Verification items for the finished model (mm, model axes). Face numbers are marked on the shaded views. Coordinates: 2 decimals unless noted, no trailing zeros. Loops run counter-clockwise (first coordinate to the right, second up) from the corner with the lowest first, then second, coordinate; pieces in that order, holes last. Notation, with made-up numbers: (10.25, 48.25) - (51.25, 48.25) arc R32 cw to (51.25, 85.25) - close; hole circle Ø11 at (26, -15). An arc over 180 degrees is marked (long way). Answer as CSV lines item,"result". Start each with the question number.
1. Release check for a two-part mould opening along Z. For the marked faces 1 and 2 record: pulls with the +Z half, pulls with the -Z half, needs draft (parallel to the pull), parting line crosses it, or undercut.
2. Cross-section at B-B (z = 637). Enter the section's corners in (x, y).
3. Cross-section at A-A (y = 382). Enter the section's corners in (x, z).
4. Gauge pin test, flat ends, axial feed: P1, Ø4, axis at x = 76.5, z = 706, coming from the +Y side; P2, Ø11.5, axis at x = 16, z = 1563, coming from the -Y side; P3, Ø7, axis at y = 16, z = 1263, coming from the +X side; P4, Ø0.6, axis at x = 68.5, z = 1, coming from the +Y side. Record the tip position at first contact, or that the pin passes through.
5. Material ranges on line 1 (Z direction, x = 16, y = 479.25); line 2 (Y direction, x = 16, z = 0.55); line 3 (Y direction, x = 16, z = 2004), recorded low to high. Write a range as [from, to].
6. Cross-section at C-C (y = 87.5). Enter the section's corners in (x, z).
```python
from build123d import *

# Parameters (mm, degrees)
EXTRUDE_1_DEPTH     = 2005
EXTRUDE_1_2_DEPTH   = 28
EXTRUDE_2_DEPTH     = 28
SKETCH_5_W          = 120
SKETCH_5_H          = 2
EXTRUDE_3_DEPTH     = 165
SKETCH_7_R          = 4.5
CUT_EXTRUDE_2_DEPTH = 10
SKETCH_8_R          = 4.5
CUT_EXTRUDE_3_DEPTH = 76
SKETCH_9_R          = 4.5
CUT_EXTRUDE_4_DEPTH = 10
SKETCH_10_R         = 4.5
CUT_EXTRUDE_5_DEPTH = 10
SKETCH_11_R         = 4.5
CUT_EXTRUDE_6_DEPTH = 16


with BuildPart() as part:
    # 草图1 → Extrude 1 (new body)
    with BuildSketch(Plane.XY):
        Polygon((0, 480), (0, 0), (150, 0), (150, 2), (2, 2), (2, 480), align=None)
    extrude(amount=EXTRUDE_1_DEPTH)

    # 草图3 → Extrude 1 2 (add)
    with BuildSketch(Plane(origin=(2, 0, 0), x_dir=(0, 0, -1), z_dir=(1, 0, 0))):
        Polygon((-2003, 2), (-2003, 478), (-2, 478), (-2, 2), (0, 2), (0, 480), (-2005, 480), (-2005, 2), align=None)
    extrude(amount=EXTRUDE_1_2_DEPTH)

    # 草图4 → 凸台-拉伸2 (add)
    with BuildSketch(Plane(origin=(0, 2, 0), x_dir=(1, 0, 0), z_dir=(0, 1, 0))):
        Polygon((148, -2003), (148, 0), (150, 0), (150, -2005), (30, -2005), (30, -2003), align=None)
    extrude(amount=EXTRUDE_2_DEPTH)

    # 草图5 → 凸台-拉伸3 (add)
    with BuildSketch(Plane(origin=(0, 2, 0), x_dir=(1, 0, 0), z_dir=(0, 1, 0))):
        with Locations((90, -1)):
            Rectangle(SKETCH_5_W, SKETCH_5_H)
    extrude(amount=EXTRUDE_3_DEPTH)

    # 草图7 → 切除-拉伸2 (cut)
    with BuildSketch(Plane.XY.offset(2)):
        with Locations((120, 153)):
            Circle(SKETCH_7_R)
        with Locations((16, 450)):
            Circle(SKETCH_7_R)
        with Locations((16, 250)):
            Circle(SKETCH_7_R)
    extrude(amount=-CUT_EXTRUDE_2_DEPTH, mode=Mode.SUBTRACT)

    # 草图8 → 切除-拉伸3 (cut)
    with BuildSketch(Plane.XZ.offset(-478)):
        with Locations((16, 30)):
            Circle(SKETCH_8_R)
        with Locations((16, 180)):
            Circle(SKETCH_8_R)
    extrude(amount=-CUT_EXTRUDE_3_DEPTH, mode=Mode.SUBTRACT)

    # 草图9 → 切除-拉伸4 (cut)
    with BuildSketch(Plane.XZ.offset(-478)):
        with Locations((16, 1975)):
            Circle(SKETCH_9_R)
        with Locations((16, 1563)):
            Circle(SKETCH_9_R)
    extrude(amount=-CUT_EXTRUDE_4_DEPTH, mode=Mode.SUBTRACT)

    # 草图10 → 切除-拉伸5 (cut)
    with BuildSketch(Plane.XY.offset(2005)):
        with Locations((16, 450)):
            Circle(SKETCH_10_R)
        with Locations((16, 197)):
            Circle(SKETCH_10_R)
        with Locations((16, 16)):
            Circle(SKETCH_10_R)
        with Locations((120, 16)):
            Circle(SKETCH_10_R)
    extrude(amount=-CUT_EXTRUDE_5_DEPTH, mode=Mode.SUBTRACT)

    # 草图11 → 切除-拉伸6 (cut)
    with BuildSketch(Plane(origin=(150, 0, 0), x_dir=(0, 0, -1), z_dir=(1, 0, 0))):
        with Locations((-30, 16)):
            Circle(SKETCH_11_R)
        with Locations((-175, 16)):
            Circle(SKETCH_11_R)
        with Locations((-1331, 16)):
            Circle(SKETCH_11_R)
        with Locations((-1263, 16)):
            Circle(SKETCH_11_R)
    extrude(amount=-CUT_EXTRUDE_6_DEPTH, mode=Mode.SUBTRACT)


solid = part.part
```
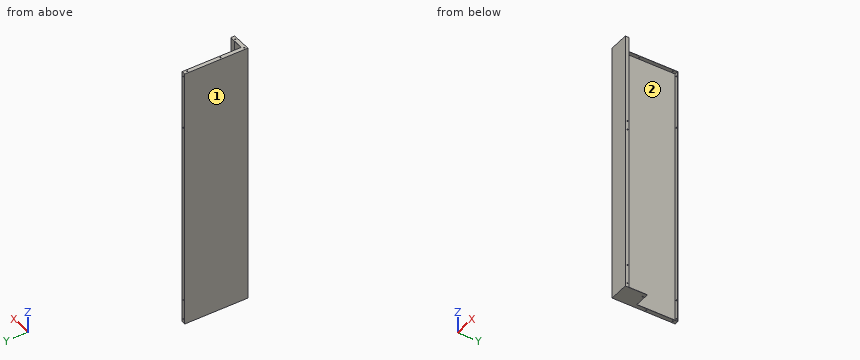
Values follow:
1,face 1,"needs draft"
1,face 2,"undercut"
2,outline,"(0, 0) - (150, 0) - (150, 30) - (148, 30) - (148, 2) - (2, 2) - (2, 478) - (30, 478) - (30, 480) - (0, 480) - close"
3,outline,"(0, 0) - (30, 0) - (30, 2) - (2, 2) - (2, 2003) - (30, 2003) - (30, 2005) - (0, 2005) - close"
4,P1,"stops at y = 2"
4,P2,"stops at y = 0"
4,P3,"stops at x = 2"
4,P4,"stops at y = 167"
5,line 1,"z = [0, 25.5], [34.5, 175.5], [184.5, 1558.5], [1567.5, 1970.5], [1979.5, 2005]"
5,line 2,"y = [0, 245.5], [254.5, 445.5], [454.5, 480]"
5,line 3,"y = [0, 11.5], [20.5, 192.5], [201.5, 445.5], [454.5, 480]"
6,outline,"(0, 0) - (150, 0) - (150, 2) - (2, 2) - (2, 2003) - (30, 2003) - (30, 2005) - (0, 2005) - close"
